from build123d import *

# Parameters (mm, degrees)
SKETCH_1_R      = 20
EXTRUDE_1_DEPTH = 150
SKETCH_2_R      = 17.5
EXTRUDE_2_DEPTH = 160
EXTRUDE_START   = 45
SKETCH_3_R      = 17.5
EXTRUDE_3_DEPTH = 45


with BuildPart() as part:
    # 草图1 → 凸台-拉伸1 (new body)
    with BuildSketch(Plane.XY):
        Circle(SKETCH_1_R)
    extrude(amount=EXTRUDE_1_DEPTH)

    # 草图2 → 凸台-拉伸2 (add)
    with BuildSketch(Plane.XY.offset(150)):
        Circle(SKETCH_2_R)
    extrude(amount=EXTRUDE_2_DEPTH)

    # 草图3 → 凸台-拉伸3 (add)
    with BuildSketch(Plane(origin=(0, 0, 0), x_dir=(-1, 0, 0), z_dir=(0, 0, -1)).offset(EXTRUDE_START)):
        with Locations(Location((0, 0, 0), (0, 0, 180))):
            Circle(SKETCH_3_R)
    extrude(amount=-EXTRUDE_3_DEPTH)


solid = part.part
Work out the finished part from the listing and answer in its coordinate system (mm). A direction names the side the tool comes from. Coordinates: 2 decimals unless noted, no trailing zeros. Write each loop counter-clockwise with the first axis right and the second up, starting at its lowest first coordinate (ties: lowest second). Pieces come first, ordered by that corner, then holes.
1. The part is cut by section A-A, the plane y = 0. Write down the section's boundary in (x, z).
Results list:
outline: (-20, 0) - (-17.5, 0) - (-17.5, -45) - (17.5, -45) - (17.5, 0) - (20, 0) - (20, 150) - (17.5, 150) - (17.5, 310) - (-17.5, 310) - (-17.5, 150) - (-20, 150) - close
2. Consider line 1 along Y through (x, z) = (-1, 284.5); line 2 along Z through (x, y) = (16.5, 7); line 3 along Y through (x, z) = (15, 0.5). Determine where each line is inside the solid, lowest interval first.
Results list:
line 1: y = -17.47 to 17.47
line 2: z = 0 to 150
line 3: y = -13.23 to 13.23
3. The part is cut by section D-D, the plane z = 120.5. Write down the section's boundary in (x, y).
Results list:
outline: circle Ø40 at (0, 0)
4. The part is cut by section C-C, the plane z = 224. Write down the section's boundary in (x, y), and give its area (3 significant figures).
Results list:
outline: circle Ø35 at (0, 0)
area: 962 mm2
5. For faces 1 (the flat face through (0, -18, 0)), 2 (the flat face through (0, 0, 310)), 3 (the flat face through (0, -18, 150)), determine the directions among +Z, -Z, +X, -X, +Y, -Y from which every point of the face is accessible in a straight line to the end or side of a thin tool.
Results list:
face 1: -Z
face 2: +Z, +X, -X, +Y, -Y
face 3: +Z
6. Flat-ended cylindrical pins translate along their axes: pin 1 (2 mm diameter, centred on x = -15.5, z = 8.5, fed in from -Y) (3 decimals); pin 2 (2 mm diameter, centred on y = 16, z = 152, fed in from +X); pin 3 (6 mm diameter, centred on y = 3.5, z = 67.5, fed in from +X); pin 4 (12 mm diameter, centred on y = 6, z = 57, fed in from -X). Find the tip coordinate at first contact, or state that the pin passes through.
Results list:
pin 1: stops at y = -13.775
pin 2: stops at x = 9.01
pin 3: stops at x = 19.99
pin 4: stops at x = -20
